Read the model definition and answer for the solid it produces. Units are mm, in the model's axes. A direction names the side the tool comes from. Round coordinates to 2 decimals unless told otherwise and drop trailing zeros. Order: outer loops, then holes, each group sorted by start corner. A loop starts at its lowest first (then second) coordinate and runs counter-clockwise, first axis right, second up. Notation, with made-up numbers: (-21, 48) -> (2, 48) arc R31 ccw to (2, 72) -> close; hole circle Ø2 at (73, 75.5). An arc over 180 degrees is marked (long way). One line per item, written item: value. Start each with the question number.
1. Flat-ended cylindrical pins translate along their axes: pin 1 Ø12 at (x, z) = (150.5, 101) entering from +Y; pin 2 Ø19.5 at (x, z) = (-150, -100) entering from -Y; pin 3 Ø7.5 at (x, z) = (-82, -3.5) entering from -Y. Find the tip coordinate at first contact, or state that the pin passes through.
2. Section C-C (x = -80) is taken. Give the vertices of the cut face in (y, z), then the cut area to 3 significant figures.
3. Section B-B (z = -100) is taken. Give the vertices of the cut face in (x, y).
4. Section A-A (x = -150) is taken. Give the vertices of the cut face in (y, z).
5. Consider line 1 (X direction, y = 13.5, z = 100); line 2 (X direction, y = 9, z = 44); line 3 (Z direction, x = -150, y = 16.25). Determine where each line is inside the solid, lowest interval first.
6. The mould has two halves that part along X. Classify faces 4 (the face through (200, 10, 2)), 5 (the face through (-143.07, 15.56, 102.87)), 6 (the face through (-3, 0, -2)): released by +X, released by -X, zero draft, split by the parting line, or undercut.
7. For faces 1 (the face through (80, 9, 1)), 2 (the face through (75.7, 18, -2.1)), 3 (the face through (-3, 10, -150)), determine the directions among +Z, -Z, +X, -X, +Y, -Y from which every point of the face is accessible in a straight line to the end or side of a thin tool.
from build123d import *

# Parameters (mm, degrees)
SKETCH1_W                                            = 400
SKETCH1_H                                            = 300
BOSS_EXTRUDE1_DEPTH                                  = 20
HOLE_SIZE_PER_SOCKET_HEAD_CAP_SCREW_TYPE_D           = 9
HOLE_SIZE_PER_SOCKET_HEAD_CAP_SCREW_TYPE_CBORE_D     = 15
HOLE_SIZE_PER_SOCKET_HEAD_CAP_SCREW_TYPE_CBORE_DEPTH = 9
SKETCH5_R                                            = 10
CUT_EXTRUDE1_DEPTH                                   = 2
HOLE_SIZE_PER_SOCKET_HEAD_CAP_SCREW_2_D              = 9
HOLE_SIZE_PER_SOCKET_HEAD_CAP_SCREW_2_CBORE_D        = 15
HOLE_SIZE_PER_SOCKET_HEAD_CAP_SCREW_2_CBORE_DEPTH    = 9
M8_TAPPED_HOLE1_D                                    = 6.8


with BuildPart() as part:
    # Sketch1 → Boss-Extrude1 (new body)
    with BuildSketch(Plane(origin=(0, 0, 0), x_dir=(1, 0, 0), z_dir=(0, 1, 0))):
        Rectangle(SKETCH1_W, SKETCH1_H)
    extrude(amount=BOSS_EXTRUDE1_DEPTH)

    # Hole size per socket head cap screw type (through all)
    with Locations(Plane(origin=(0, 20, 0), x_dir=(1, 0, 0), z_dir=(0, 1, 0))):
        with Locations((-150, 100), (-150, -100), (150, 100), (150, -100)):
            CounterBoreHole(HOLE_SIZE_PER_SOCKET_HEAD_CAP_SCREW_TYPE_D / 2, HOLE_SIZE_PER_SOCKET_HEAD_CAP_SCREW_TYPE_CBORE_D / 2, HOLE_SIZE_PER_SOCKET_HEAD_CAP_SCREW_TYPE_CBORE_DEPTH)

    # Sketch5 → Cut-Extrude1 (cut)
    with BuildSketch(Plane(origin=(0, 20, 0), x_dir=(1, 0, 0), z_dir=(0, 1, 0))):
        with Locations(Location((-80, 4.166410727, 0), (0, 0, 270))):
            Circle(SKETCH5_R)
        with Locations(Location((80, 4.166410727, 0), (0, 0, 270))):
            Circle(SKETCH5_R)
    extrude(amount=-CUT_EXTRUDE1_DEPTH, mode=Mode.SUBTRACT)

    # Hole size per socket head cap screw  2 (through all)
    with Locations(Plane(origin=(0, 0, 0), x_dir=(-1, 0, 0), z_dir=(0, -1, 0))):
        with Locations((80, 4.166410727), (-80, 4.166410727)):
            CounterBoreHole(HOLE_SIZE_PER_SOCKET_HEAD_CAP_SCREW_2_D / 2, HOLE_SIZE_PER_SOCKET_HEAD_CAP_SCREW_2_CBORE_D / 2, HOLE_SIZE_PER_SOCKET_HEAD_CAP_SCREW_2_CBORE_DEPTH)

    # M8 Tapped Hole1 (through all)
    with Locations(Plane(origin=(0, 20, 0), x_dir=(1, 0, 0), z_dir=(0, 1, 0))):
        with Locations((-35, 50), (-35, -44), (50, -44), (50, 50)):
            Hole(M8_TAPPED_HOLE1_D / 2)


solid = part.part
Answer:
1. pin 1: y = 11
1. pin 2: y = 0
1. pin 3: y = 9
2. outline: (0, -150) -> (20, -150) -> (20, -14.17) -> (18, -14.17) -> (18, -8.67) -> (9, -8.67) -> (9, -11.67) -> (0, -11.67) -> close; (0, 3.33) -> (9, 3.33) -> (9, 0.33) -> (18, 0.33) -> (18, 5.83) -> (20, 5.83) -> (20, 150) -> (0, 150) -> close
2. area: 5,740 mm^2
3. outline: (-200, 0) -> (-154.5, 0) -> (-154.5, 11) -> (-157.5, 11) -> (-157.5, 20) -> (-200, 20) -> close; (-145.5, 0) -> (145.5, 0) -> (145.5, 11) -> (142.5, 11) -> (142.5, 20) -> (-142.5, 20) -> (-142.5, 11) -> (-145.5, 11) -> close; (154.5, 0) -> (200, 0) -> (200, 20) -> (157.5, 20) -> (157.5, 11) -> (154.5, 11) -> close
4. outline: (0, -150) -> (20, -150) -> (20, -107.5) -> (11, -107.5) -> (11, -104.5) -> (0, -104.5) -> close; (0, -95.5) -> (11, -95.5) -> (11, -92.5) -> (20, -92.5) -> (20, 92.5) -> (11, 92.5) -> (11, 95.5) -> (0, 95.5) -> close; (0, 104.5) -> (11, 104.5) -> (11, 107.5) -> (20, 107.5) -> (20, 150) -> (0, 150) -> close
5. line 1: -200 to -157.5, -142.5 to 142.5, 157.5 to 200
5. line 2: -200 to -38.4, -31.6 to 46.6, 53.4 to 200
5. line 3: -150 to -107.5, -92.5 to 92.5, 107.5 to 150
6. face 4: released by +X
6. face 5: undercut
6. face 6: zero draft
7. face 1: -Y
7. face 2: +Y
7. face 3: -Z, +X, -X, +Y, -Y
